Verification items for the finished model (mm, model axes). Face numbers are marked on the shaded views. A direction names the side the tool comes from. Round coordinates to 2 decimals unless told otherwise and drop trailing zeros. Loops run counter-clockwise (first coordinate to the right, second up) from the corner with the lowest first, then second, coordinate; pieces in that order, holes last.
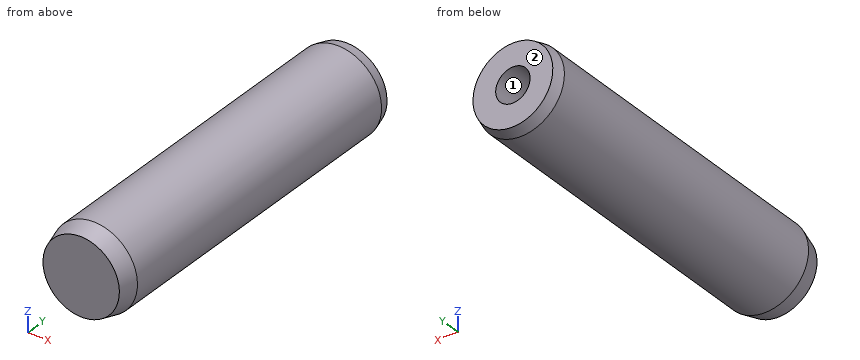
from build123d import *

# Parameters (mm, degrees)
SKETCH1_R             = 6
BOSS_EXTRUDE1_DEPTH   = 25
M6_TAPPED_HOLE1_D     = 4.8
M6_TAPPED_HOLE1_DEPTH = 20
M6_TAPPED_HOLE1_TIP   = 1.385640646
CHAMFER1_SIZE         = 1.6
CHAMFER1_SIZE2        = 0.428718708
CHAMFER2_SIZE         = 2.5
CHAMFER2_SIZE2        = 0.669872981


with BuildPart() as part:
    # Sketch1 → Boss-Extrude1 (new, symmetric)
    with BuildSketch(Plane(origin=(0, 0, 0), x_dir=(1, 0, 0), z_dir=(0, 1, 0))):
        with Locations(Location((0, 0, 0), (0, 0, 270))):
            Circle(SKETCH1_R)
    extrude(amount=BOSS_EXTRUDE1_DEPTH, both=True)

    # M6 Tapped Hole1
    with Locations(Plane(origin=(0, 25, 0), x_dir=(1, 0, 0), z_dir=(0, 1, 0))):
        with Locations((0, 0)):
            Hole(M6_TAPPED_HOLE1_D / 2, depth=M6_TAPPED_HOLE1_DEPTH)
            with Locations((0, 0, -(M6_TAPPED_HOLE1_DEPTH + M6_TAPPED_HOLE1_TIP / 2))):  # 120° drill point
                Cone(0, M6_TAPPED_HOLE1_D / 2, M6_TAPPED_HOLE1_TIP, mode=Mode.SUBTRACT)

    # Chamfer1
    chamfer1_edges = [part.edges().sort_by_distance(p)[0] for p in [
        (0, 25, -6),
    ]]
    chamfer1_side = [part.faces().sort_by_distance(p)[0] for p in [
        (0, 0, -6),
    ]]
    chamfer(chamfer1_edges, length=CHAMFER1_SIZE, length2=CHAMFER1_SIZE2, reference=chamfer1_side[0])

    # Chamfer2
    chamfer2_edges = [part.edges().sort_by_distance(p)[0] for p in [
        (0, -25, -6),
    ]]
    chamfer2_side = [part.faces().sort_by_distance(p)[0] for p in [
        (0, -0.8, -6),
    ]]
    chamfer(chamfer2_edges, length=CHAMFER2_SIZE, length2=CHAMFER2_SIZE2, reference=chamfer2_side[0])


solid = part.part
1. Scan lines: L1, parallel to Z at x = -0.75, y = 22; L2, parallel to Z at x = 0.25, y = 21; L3, parallel to X at y = -2.5, z = 2.25. Record each from-to range of solid material in increasing order.
2. Section check B-B (y = -10.5). Enter the section's corners in (x, z).
3. Tool access check on the marked faces 1 and 2. Record the directions out of +Z, -Z, +X, -X, +Y, -Y that give a thin tool (end or side, any length) a straight path to the whole face; none if there is none.
4. Gauge pin test, flat ends, axial feed: P1, Ø1, axis at x = -1, y = -11, coming from the -Z side; P2, Ø2, axis at x = -4, y = 15, coming from the -Z side; P3, Ø2, axis at x = 3, y = 5, coming from the -Z side. Record the tip position at first contact, or that the pin passes through.
5. Section check A-A (y = 10.5). Enter the section's corners in (x, z).
Taken from the geometry:
1. L1: z = -5.95 to -2.28, 2.28 to 5.95
1. L2: z = -5.99 to -2.39, 2.39 to 5.99
1. L3: x = -5.56 to 5.56
2. outline: circle Ø12 at (0, 0)
3. face 1: +Y
3. face 2: +Z, -Z, +X, -X, +Y
4. P1: stops at z = -5.98
4. P2: stops at z = -5.2
4. P3: stops at z = -5.66
5. outline: circle Ø12 at (0, 0); hole circle Ø4.8 at (0, 0)
